Verification items for the finished model (mm, model axes). Face numbers are marked on the shaded views. A direction names the side the tool comes from. Give positions to 0.01 mm unless a question says otherwise; leave off trailing zeros. Loops run counter-clockwise (first coordinate to the right, second up) from the corner with the lowest first, then second, coordinate; pieces in that order, holes last. Notation, with made-up numbers: (-5, 75.5) - (23, 75.5) arc R8 cw to (23, 79.5) - close; hole circle Ø6 at (50, -16). An arc over 180 degrees is marked (long way). One line per item, written item: value. Start each with the question number.
1. Sectioned sample at D-D (x = -5). Record the cut outline in (y, z).
2. Sectioned sample at B-B (x = 0). Record the cut outline in (y, z).
3. Access from +Z, -Z, +X, -X, +Y, -Y to the whole of each face (thin tool, end or side, straight path). Record for the marked faces 4, 5 and 6.
4. Sectioned sample at C-C (y = 4). Record the cut outline in (x, z).
5. Mould release check, pull along X, two halves, no side actions. Record for the marked faces 1, 2 and 3: pulls with the +X half, pulls with the -X half, needs draft (parallel to the pull), parting line crosses it, or undercut.
6. Gauge pin test, flat ends, axial feed: pin 1 (2.5 mm diameter, centred on y = 4.5, z = 9.5, fed in from -X); pin 2 (2.5 mm diameter, centred on x = 10.5, y = 6.5, fed in from -Z); pin 3 (2.5 mm diameter, centred on y = 5.5, z = -9.5, fed in from +X). Record the tip position at first contact, or that the pin passes through.
7. Scan lines: L1, parallel to Y at x = 6, z = -9; L2, parallel to Z at x = 2.5, y = 4.75. Record each from-to range of solid material in increasing order. Write a range as [from, to].
8. Sectioned sample at A-A (z = 0). Record the cut outline in (x, y), plus the area to 3 significant figures.
from build123d import *

# Parameters (mm, degrees)
SKETCH1_R           = 16
BOSS_EXTRUDE2_DEPTH = 2
SKETCH4_W           = 8
SKETCH4_H           = 8
BOSS_EXTRUDE7_DEPTH = 8
SKETCH5_R           = 16
BOSS_EXTRUDE8_DEPTH = 2


with BuildPart() as part:
    # Sketch1 → Boss-Extrude2 (new body)
    with BuildSketch(Plane(origin=(0, 0, 0), x_dir=(1, 0, 0), z_dir=(0, 1, 0))):
        with Locations(Location((0, 0, 0), (0, 0, 270))):
            Circle(SKETCH1_R)
    extrude(amount=BOSS_EXTRUDE2_DEPTH)

    # Sketch4 → Boss-Extrude7 (add)
    with BuildSketch(Plane(origin=(0, 2, 0), x_dir=(1, 0, 0), z_dir=(0, 1, 0))):
        with Locations((-10, 0)):
            Rectangle(SKETCH4_W, SKETCH4_H)
        with Locations((0, -10)):
            Rectangle(SKETCH4_W, SKETCH4_H)
        with Locations((0, 10)):
            Rectangle(SKETCH4_W, SKETCH4_H)
        with Locations((10, 0)):
            Rectangle(SKETCH4_W, SKETCH4_H)
    extrude(amount=BOSS_EXTRUDE7_DEPTH)

    # Sketch5 → Boss-Extrude8 (add)
    with BuildSketch(Plane(origin=(0, 10, 0), x_dir=(-1, 0, 0), z_dir=(0, -1, 0))):
        with Locations(Location((0, 0, 0), (0, 0, 270))):
            Circle(SKETCH5_R)
    extrude(amount=-BOSS_EXTRUDE8_DEPTH)


solid = part.part
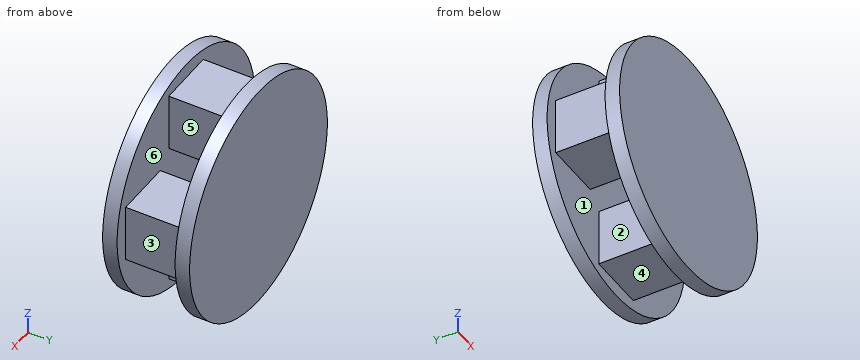
Results are:
1. outline: (0, -15.2) - (2, -15.2) - (2, 15.2) - (0, 15.2) - close; (10, -15.2) - (12, -15.2) - (12, 15.2) - (10, 15.2) - close
2. outline: (0, -16) - (2, -16) - (2, -14) - (10, -14) - (10, -16) - (12, -16) - (12, 16) - (10, 16) - (10, 14) - (2, 14) - (2, 16) - (0, 16) - close; hole (2, -6) - (10, -6) - (10, 6) - (2, 6) - close
3. face 4: -Z, +X, -X
3. face 5: +Z, -Z, +X
3. face 6: none
4. outline: (-14, -4) - (-6, -4) - (-6, 4) - (-14, 4) - close; (-4, -14) - (4, -14) - (4, -6) - (-4, -6) - close; (-4, 6) - (4, 6) - (4, 14) - (-4, 14) - close; (6, -4) - (14, -4) - (14, 4) - (6, 4) - close
5. face 1: undercut
5. face 2: pulls with the -X half
5. face 3: pulls with the +X half
6. pin 1: stops at x = -4
6. pin 2: stops at z = -4
6. pin 3: stops at x = 4
7. L1: y = [0, 2], [10, 12]
7. L2: z = [-14, -6], [6, 14]
8. outline: (-16, 0) - (16, 0) - (16, 2) - (14, 2) - (14, 10) - (16, 10) - (16, 12) - (-16, 12) - (-16, 10) - (-14, 10) - (-14, 2) - (-16, 2) - close; hole (-6, 2) - (6, 2) - (6, 10) - (-6, 10) - close
8. area: 256 mm^2
